Input: dimensioned drawing with shaded views. Units: mm. Origin: part minimum x, y, z. A direction names the side the tool comes from. Give positions to 0.01 mm unless a question says otherwise; leave off trailing zeros. Write each loop counter-clockwise with the first axis right and the second up, starting at its lowest first coordinate (ties: lowest second). Pieces come first, ordered by that corner, then holes. Notation, with made-up numbers: (11, 42.5) - (55, 42.5) arc R18 ccw to (55, 68.5) - close; hole circle Ø6 at (27.25, -27). An arc over 180 degrees is marked (long way). Answer as a JSON object with one key per item and string values. Group by question number.
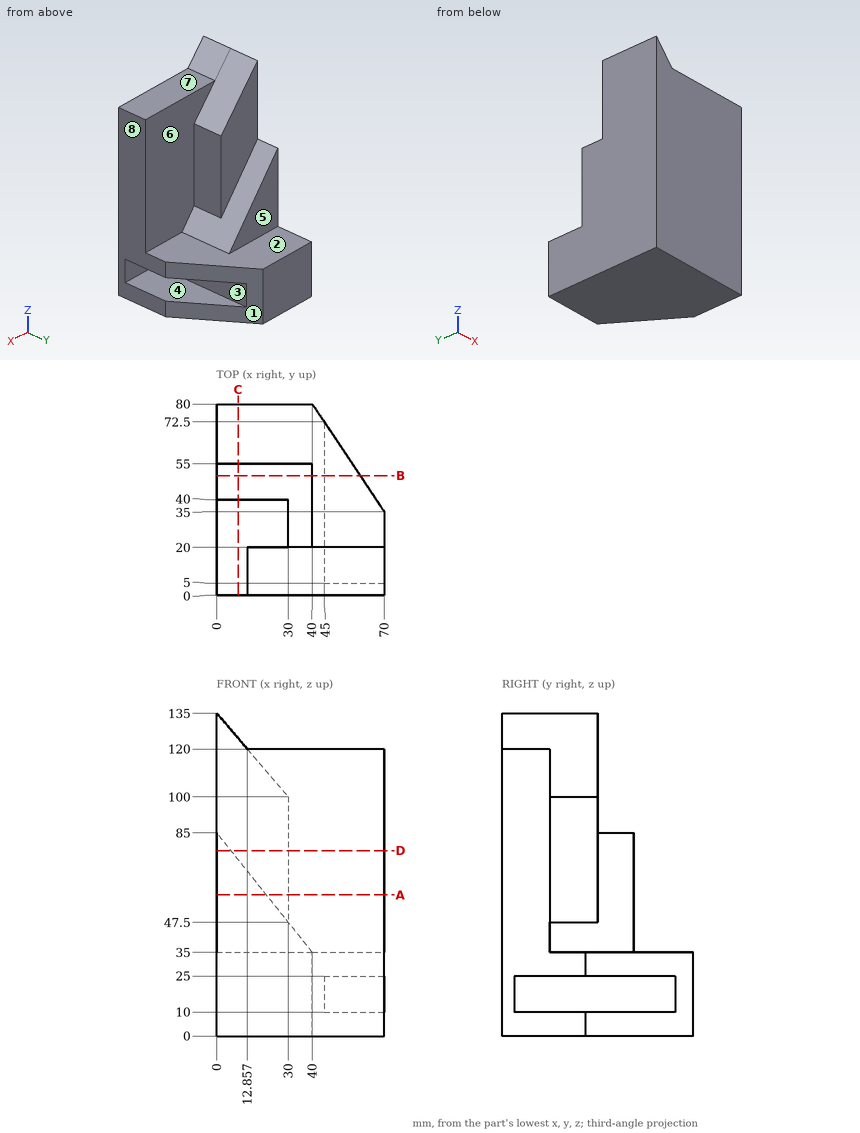
Q1. Draft query along Z for the marked faces 1, 2 and 3. Return one class per face: released by +Z, released by -Z, zero draft, split by the parting line, or undercut.
Q2. Ray query, probe 1 along X at (y, z) = (51, 14); probe 2 along Y at (x, z) = (44, 101.5); probe 3 along Z at (x, y) = (52, 50). Return the intervals inside material, ascending. Write a range as [from, to].
Q3. Reachability of the marked faces 4, 5, 6, 7 and 8 from +Z, -Z, +X, -X, +Y, -Y: full face, straight path, thin tool, end or side. Return the list, or none.
Q4. Section A-A on z = 59. Return the cut outline in (x, y), then the cut area to 3 significant figures.
Q5. Section B-B on y = 50. Return the cut outline in (x, z).
Q6. Section D-D on z = 77.5. Return the cut outline in (x, y).
Q7. First-contact query: pin 1 Ø12 at (x, z) = (55.5, 17) entering from +Y; pin 2 Ø12 at (x, z) = (47, 60) entering from +Y; pin 3 Ø1.5 at (x, y) = (37, 41.5) entering from -Z; pin 4 Ø2 at (y, z) = (25.5, 15.5) entering from +X. Flat tips, straight axial feed; report the tip coordinate or a pass-through.
Q8. Section C-C on x = 9. Return the cut outline in (y, z).
Taken from the geometry:
{
 "1": {"face 1": "zero draft", "face 2": "released by +Z", "face 3": "undercut"},
 "2": {"probe 1": "x = [0, 45]", "probe 2": "y = [0, 20]", "probe 3": "z = [0, 10], [25, 35]"},
 "3": {"face 4": "+X, +Y", "face 5": "+Z, +X, -X, +Y", "face 6": "+Z, +X, +Y", "face 7": "+Z, +X, +Y, -Y", "face 8": "+Z, -Z, +X, +Y, -Y"},
 "4": {"outline": "(0, 0) - (70, 0) - (70, 20) - (30, 20) - (30, 40) - (20.8, 40) - (20.8, 55) - (0, 55) - close", "area": "2,310 mm²"},
 "5": {"outline": "(0, 0) - (60, 0) - (60, 10) - (45, 10) - (45, 25) - (60, 25) - (60, 35) - (40, 35) - (0, 85) - close"},
 "6": {"outline": "(0, 0) - (70, 0) - (70, 20) - (30, 20) - (30, 40) - (6, 40) - (6, 55) - (0, 55) - close"},
 "7": {"pin 1": "stops at y = 5", "pin 2": "stops at y = 20", "pin 3": "stops at z = 0", "pin 4": "stops at x = 45"},
 "8": {"outline": "(0, 0) - (80, 0) - (80, 35) - (55, 35) - (55, 73.75) - (40, 73.75) - (40, 124.5) - (0, 124.5) - close"}
}
